Design review of the part built by this model. Coordinates are the model's own, in mm. Give positions to 0.01 mm unless a question says otherwise; leave off trailing zeros. Order: outer loops, then holes, each group sorted by start corner. A loop starts at its lowest first (then second) coordinate and runs counter-clockwise, first axis right, second up. Notation, with made-up numbers: (47, -5.75) -> (83, -5.75) arc R26 cw to (83, 30.25) -> close; hole circle Ø8 at (4.5, -29). An arc over 180 degrees is marked (long way). One line per item, written item: value. Start each with the question number.
1) Wall thickness on line 1 along Z through (x, y) = (44.5, 6.25); line 2 along Y through (x, z) = (-6, -4.5); line 3 along Z through (x, y) = (312.5, 8): over which ranges is each line inside the solid? List them lowest first. Write a range as from..to.
2) Consider section A-A (y = 3.5). State how many separate pieces and enclosed holes the cut face has, plus the area to 3 significant figures.
3) Consider section C-C (x = 209.5). State the section outline as (y, z) points, plus the area to 3 significant figures.
4) For pin 1 (1.5 mm diameter, centred on x = 368.5, z = -6, fed in from -Y); pin 2 (1.5 mm diameter, centred on y = 4.5, z = 3.5, fed in from +X); pin 3 (1.5 mm diameter, centred on y = 5.5, z = -4.5, fed in from +X), all flat-tipped, find the tip position at first contact; note any pin that passes through.
from build123d import *

# Parameters (mm, degrees)
BOSS_EXTRUDE1_DEPTH = 9
M8_TAPPED_HOLE1_D   = 6.8
LPATTERN1_COUNT     = 19
LPATTERN1_PITCH     = 30
CUT_EXTRUDE1_START  = -200
CUT_EXTRUDE1_DEPTH  = 705.20277905


with BuildPart() as part:
    # Sketch1 → Boss-Extrude1 (new body)
    with BuildSketch(Plane(origin=(0, 0, 0), x_dir=(1, 0, 0), z_dir=(0, 1, 0))):
        with BuildLine():
            Line((-90.976744186, 10), (494.023255814, 10))
            ThreePointArc((494.023255814, 10), (504.023255814, 0), (494.023255814, -10))
            Line((494.023255814, -10), (-90.976744186, -10))
            ThreePointArc((-90.976744186, -10), (-100.976744186, 0), (-90.976744186, 10))
        make_face()
    extrude(amount=BOSS_EXTRUDE1_DEPTH)

    # M8 Tapped Hole1 (through all)
    with Locations(Plane(origin=(0, 9, 0), x_dir=(1, 0, 0), z_dir=(0, 1, 0))):
        with Locations((-75.976744186, 0)):
            m8_tapped_hole1 = Hole(M8_TAPPED_HOLE1_D / 2)

    # LPattern1: M8 Tapped Hole1 ×19
    with Locations(*[(i * LPATTERN1_PITCH, 0, 0) for i in range(1, LPATTERN1_COUNT)]):
        add(m8_tapped_hole1, mode=Mode.SUBTRACT)

    # Sketch4 → Cut-Extrude1 (cut, through all)
    with BuildSketch(Plane(origin=(0, 0, 0), x_dir=(0, 0, -1), z_dir=(1, 0, 0)).offset(CUT_EXTRUDE1_START)):
        Polygon((4, 0), (14, 0), (14, 2.216946626), align=None)
        Polygon((-14, 2.216946626), (-14, 0), (-4, 0), align=None)
    extrude(amount=CUT_EXTRUDE1_DEPTH, mode=Mode.SUBTRACT)


solid = part.part
Checked values:
1. line 1: z = -10..-3.37, 3.37..10
1. line 2: y = 0.11..9
1. line 3: z = -10..-3.04, 3.04..10
2. separate pieces: 1
2. enclosed holes: 19
2. area: 11,300 mm^2
3. outline: (0, -4) -> (1.33, -10) -> (9, -10) -> (9, 10) -> (1.33, 10) -> (0, 4) -> close
3. area: 172 mm^2
4. pin 1: stops at y = 0.28
4. pin 2: stops at x = 503.64
4. pin 3: stops at x = 503.29
